Part model, mm, in its own coordinate system. Coordinates: 2 decimals unless noted, no trailing zeros. Loops run counter-clockwise (first coordinate to the right, second up) from the corner with the lowest first, then second, coordinate; pieces in that order, holes last. Notation, with made-up numbers: (59, -28.75) - (107, -28.75) arc R15 cw to (107, -16.75) - close; hole circle Ø11 at (9, 59). An arc over 180 degrees is marked (long way). Use a Markdown table: item, result. Add a question column.
1. Pull direction Y, two halves, no side cores. Call faces 1 (the flat face through (-6, 1, 0.5)), 2 (the cylindrical face through (-225.5, -12.4, 0)): pulls with the +Y half, pulls with the -Y half, needs draft (parallel to the pull), parting line crosses it, or undercut.
2. Wall check: probe 1 along X at (y, z) = (-41, -0.3); probe 2 along X at (y, z) = (17.5, 0.45); probe 3 along X at (y, z) = (-39.5, -0.35). Give the ranges that are in metal, low to high. Write a range as [from, to].
3. Band-saw the part on B-B, the plane x = 180. Give the cut face in (y, z), plus the area to 3 significant figures.
4. Band-saw the part on A-A, the plane y = -17.5. Give the cut face in (x, z), plus the area to 3 significant figures.
from build123d import *

# Parameters (mm, degrees)
SKETCH1_W                = 920
SKETCH1_H                = 1
EXTRUDE1_DEPTH           = 52.5
SKETCH2_R                = 7.5
CUT_EXTRUDE1_DEPTH       = 463.987310841
M5_CLEARANCE_HOLE1_D     = 6
M5_CLEARANCE_HOLE1_DEPTH = 7
M5_CLEARANCE_HOLE1_TIP   = 1.802581857


with BuildPart() as part:
    # Sketch1 → Extrude1 (new, symmetric)
    with BuildSketch(Plane(origin=(0, 0, 0), x_dir=(1, 0, 0), z_dir=(0, 1, 0))):
        Rectangle(SKETCH1_W, SKETCH1_H)
    extrude(amount=EXTRUDE1_DEPTH, both=True)

    # Sketch2 → Cut-Extrude1 (cut, through all)
    with BuildSketch(Plane.XY.offset(0.5)):
        with Locations((-220, -17.5)):
            Circle(SKETCH2_R)
        with Locations((180, -17.5)):
            Circle(SKETCH2_R)
    extrude(amount=-CUT_EXTRUDE1_DEPTH, mode=Mode.SUBTRACT)

    # M5 Clearance Hole1
    with Locations(Plane.XY.offset(0.5)):
        with Locations((-420, -41.5), (-140, -41.5), (140, -41.5), (-365, 18.5), (330, 18.5), (420, -41.5)):
            Hole(M5_CLEARANCE_HOLE1_D / 2, depth=M5_CLEARANCE_HOLE1_DEPTH)
            with Locations((0, 0, -(M5_CLEARANCE_HOLE1_DEPTH + M5_CLEARANCE_HOLE1_TIP / 2))):  # 118° drill point
                Cone(0, M5_CLEARANCE_HOLE1_D / 2, M5_CLEARANCE_HOLE1_TIP, mode=Mode.SUBTRACT)


solid = part.part
Geometry check:
| question | item | result |
|---|---|---|
| 1 | face 1 | needs draft |
| 1 | face 2 | undercut |
| 2 | probe 1 | x = [-460, -422.96], [-417.04, -142.96], [-137.04, 137.04], [142.96, 417.04], [422.96, 460] |
| 2 | probe 2 | x = [-460, -367.83], [-362.17, 327.17], [332.83, 460] |
| 2 | probe 3 | x = [-460, -422.24], [-417.76, -142.24], [-137.76, 137.76], [142.24, 417.76], [422.24, 460] |
| 3 | outline | (-52.5, -0.5) - (-25, -0.5) - (-25, 0.5) - (-52.5, 0.5) - close; (-10, -0.5) - (52.5, -0.5) - (52.5, 0.5) - (-10, 0.5) - close |
| 3 | area | 90.0 mm^2 |
| 4 | outline | (-460, -0.5) - (-227.5, -0.5) - (-227.5, 0.5) - (-460, 0.5) - close; (-212.5, -0.5) - (172.5, -0.5) - (172.5, 0.5) - (-212.5, 0.5) - close; (187.5, -0.5) - (460, -0.5) - (460, 0.5) - (187.5, 0.5) - close |
| 4 | area | 890 mm^2 |
